```python
from build123d import *

# Parameters (mm, degrees)
SKETCH1_W           = 116
SKETCH1_H           = 176
BOSS_EXTRUDE1_DEPTH = 30
SKETCH3_R           = 5.055
CUT_EXTRUDE1_DEPTH  = 188.723200484


with BuildPart() as part:
    # Sketch1 → Boss-Extrude1 (new body)
    with BuildSketch(Plane.XY):
        Rectangle(SKETCH1_W, SKETCH1_H)
    extrude(amount=BOSS_EXTRUDE1_DEPTH)

    # Sketch3 → Cut-Extrude1 (cut, through all)
    with BuildSketch(Plane(origin=(0, 88, 0), x_dir=(1, 0, 0), z_dir=(0, 1, 0))):
        with Locations(Location((0, -15, 0), (0, 0, 180))):
            Circle(SKETCH3_R)
    extrude(amount=-CUT_EXTRUDE1_DEPTH, mode=Mode.SUBTRACT)


solid = part.part
```
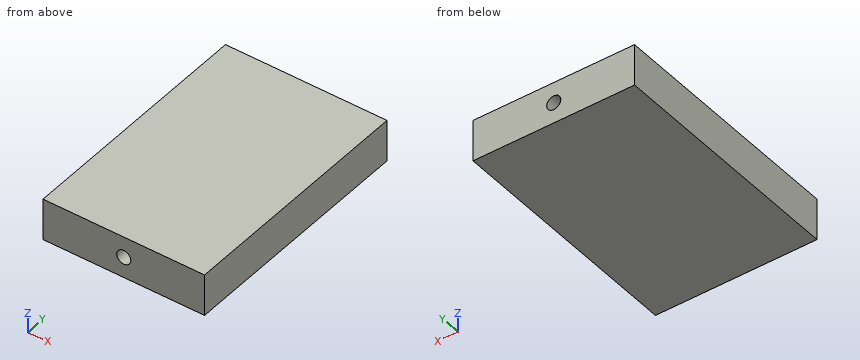
Here's how the part is built. I have some questions about the finished solid (model axes, mm). Give positions to 0.01 mm unless a question says otherwise; leave off trailing zeros. Write each loop counter-clockwise with the first axis right and the second up, starting at its lowest first coordinate (ties: lowest second). Pieces come first, ordered by that corner, then holes. Notation, with made-up numbers: M 71.25,-29.75 L 87.25,-29.75 A35 ccw 87.25,3.25 Z; hole C 7,-30 d8. An arc over 180 degrees is marked long. Put each result on its own line as item: value. Start each with the question number.
Item 1: If we section it at C-C, the plane y = -0.5: Write out the boundary of the cut face in (x, z) (3 decimals), then the cut area to 3 significant figures.
Item 2: I need wall thicknesses on L1, parallel to Z at x = 0, y = 30 (3 decimals); L2, parallel to Z at x = -4.5, y = 75; L3, parallel to X at y = 59, z = 19.5. Which ranges of each line are inside material? Lowest first, please. Write a range as from..to.
Item 3: Will this pin go through, and if not, where does the flat tip stop? pin 1 (6 mm diameter, centred on x = 0, z = 15, fed in from +Y).
Item 4: If we section it at B-B, the plane z = 15: Write out the boundary of the cut face in (x, y) (3 decimals).
Item 5: If we section it at A-A, the plane x = 0: Write out the boundary of the cut face in (y, z) (3 decimals), then the cut area to 3 significant figures.
Values:
1. outline: M -58,0 L 58,0 L 58,30 L -58,30 Z; hole C 0,15 d10.11
1. area: 3,400 mm²
2. L1: 0..9.945, 20.055..30
2. L2: 0..12.7, 17.3..30
2. L3: -58..-2.3, 2.3..58
3. pin 1: through
4. outline: M -58,-88 L -5.055,-88 L -5.055,88 L -58,88 Z; M 5.055,-88 L 58,-88 L 58,88 L 5.055,88 Z
5. outline: M -88,0 L 88,0 L 88,9.945 L -88,9.945 Z; M -88,20.055 L 88,20.055 L 88,30 L -88,30 Z
5. area: 3,500 mm²
